Input: part model. Units: mm. Frame: model coordinates. Face numbers are marked on the shaded views. A direction names the side the tool comes from. Round coordinates to 2 decimals unless told otherwise and drop trailing zeros. Write each loop counter-clockwise with the first axis right and the second up, starting at its lowest first coordinate (ties: lowest second). Pieces come first, ordered by that corner, then holes. Notation, with made-up numbers: M 87.5,88 L 126.5,88 A16 ccw 126.5,93 Z; hole C 5.25,39 d7. An arc over 180 degrees is marked long. Answer as CSV lines item,"result". Start each with the question number.
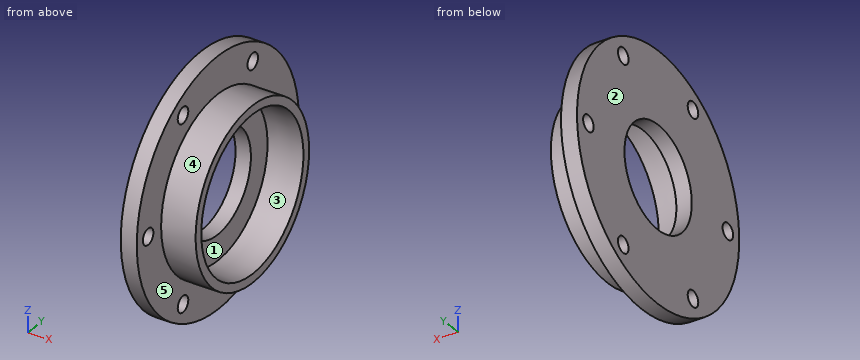
```python
from build123d import *

# Parameters (mm, degrees)
SKETCH2_R          = 6.5
CUT_EXTRUDE1_DEPTH = 145.166570328
CIRPATTERN1_COUNT  = 6
SKETCH3_R          = 41.5
CUT_EXTRUDE2_DEPTH = 148.244694302
DRAFT1_ANGLE       = 2


with BuildPart() as part:
    # Sketch1 → Revolve1 (revolve)
    with BuildSketch(Plane.XY, mode=Mode.PRIVATE) as revolve1_sk:
        Polygon((0, 0), (0, 100), (13, 100), (13, 70), (41, 70), (41, 62), (12.495221111, 62), (12.495221111, 0), align=None)
    revolve(revolve1_sk.sketch.rotate(Axis((0, 0, 0), (1, 0, 0)), 90), axis=Axis((0, 0, 0), (1, 0, 0)))

    # Sketch2 → Cut-Extrude1 (cut, through all)
    with BuildSketch(Plane(origin=(13, 0, 0), x_dir=(0, 0, -1), z_dir=(1, 0, 0))):
        with Locations((0, 86)):
            Circle(SKETCH2_R)
    cut_extrude1 = extrude(amount=-CUT_EXTRUDE1_DEPTH, mode=Mode.SUBTRACT)

    # CirPattern1: Cut-Extrude1 ×6 about axis
    cirpattern1_axis = Axis((0, 0, 0), (1, 0, 0))
    for i in range(1, CIRPATTERN1_COUNT):
        add(cut_extrude1.rotate(cirpattern1_axis, i * 360 / CIRPATTERN1_COUNT), mode=Mode.SUBTRACT)

    # Sketch3 → Cut-Extrude2 (cut, through all)
    with BuildSketch(Plane.ZY):
        Circle(SKETCH3_R)
    extrude(amount=-CUT_EXTRUDE2_DEPTH, mode=Mode.SUBTRACT)

    # Draft1
    draft1_faces = [part.faces().sort_by_distance(p)[0] for p in [
        (26.747610556, 0, -62),
    ]]
    draft(draft1_faces, Plane(origin=(12.495221111, 62, 0), x_dir=(0, 0, 1), z_dir=(1, 0, 0)), DRAFT1_ANGLE)


solid = part.part
```
Item 1: Access query for the marked faces 1 and 2. Directions: +Z, -Z, +X, -X, +Y, -Y. A direction counts if a zero-diameter tool reaches every point of the face in a straight line with its end or side. Return the directions, or none.
Item 2: Cut plane D-D, the plane y = -86. Return loops of the section in (x, z), plus the area to 3 significant figures.
Item 3: Pin query (flat end, axial travel): pin 1 Ø10 at (x, y) = (7, -31.5) entering from -Z; pin 2 Ø15 at (y, z) = (43, -74.48) entering from +X; pin 3 Ø12 at (x, y) = (22.5, -58) entering from -Z. Return the tip coordinate at first contact, or that it passes through.
Item 4: Draft query along Z for the marked faces 3, 4 and 5. Return one class per face: +Z half, -Z half, draft (parallel to the pull), parting line (faces both ways), or undercut.
Item 5: Cut plane A-A, the plane z = 0. Return loops of the section in (x, y).
Item 6: Cut plane B-B, the plane y = 0. Return loops of the section in (x, z), plus the area to 3 significant figures.
Item 7: Cut plane C-C, the plane x = 8. Return loops of the section in (y, z).
Item 8: Line query: line 1 (Y direction, x = 7, z = 0); line 2 (Y direction, x = 8.5, z = -74); line 3 (X direction, y = -71, z = -26.5). Output: solid intervals per line, ascending. Write a range as [from, to].
Results list:
1,face 1,"+X"
1,face 2,"+Z, -Z, -X, +Y, -Y"
2,outline,"M 0,-51.03 L 13,-51.03 L 13,-6.5 L 0,-6.5 Z; M 0,6.5 L 13,6.5 L 13,51.03 L 0,51.03 Z"
2,area,"1,160 mm²"
3,pin 1,"z = -96.42"
3,pin 2,"x = 13"
3,pin 3,"z = -46.86"
4,face 3,"undercut"
4,face 4,"parting line"
4,face 5,"draft"
5,outline,"M 0,-100 L 13,-100 L 13,-92.5 L 0,-92.5 Z; M 0,-79.5 L 13,-79.5 L 13,-70 L 41,-70 L 41,-63 L 12.5,-62 L 12.5,-41.5 L 0,-41.5 Z; M 0,41.5 L 12.5,41.5 L 12.5,62 L 41,63 L 41,70 L 13,70 L 13,79.5 L 0,79.5 Z; M 0,92.5 L 13,92.5 L 13,100 L 0,100 Z"
6,outline,"M 0,-100 L 13,-100 L 13,-70 L 41,-70 L 41,-63 L 12.5,-62 L 12.5,-41.5 L 0,-41.5 Z; M 0,41.5 L 12.5,41.5 L 12.5,62 L 41,63 L 41,70 L 13,70 L 13,100 L 0,100 Z"
6,area,"1,920 mm²"
7,outline,"C 0,0 d200; hole C -86,0 d13; hole C -43,-74.48 d13; hole C -43,74.48 d13; hole C 0,0 d83; hole C 43,-74.48 d13; hole C 43,74.48 d13; hole C 86,0 d13"
8,line 1,"[-100, -92.5], [-79.5, -41.5], [41.5, 79.5], [92.5, 100]"
8,line 2,"[-67.26, -49.48], [-36.52, 36.52], [49.48, 67.26]"
8,line 3,"[0, 13]"
